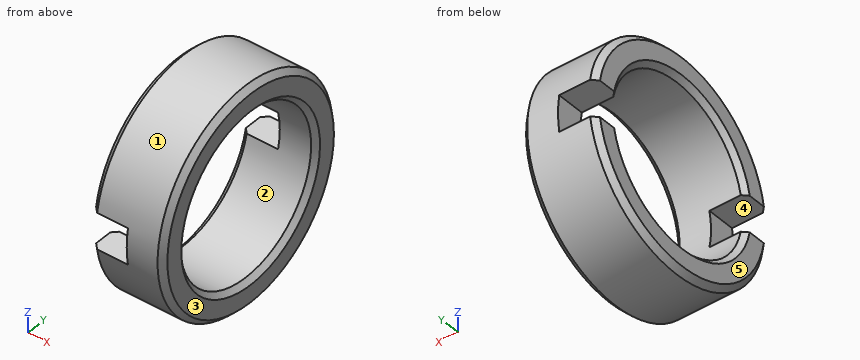
from build123d import *

# Parameters (mm, degrees)
CUT_EXTRUDE_1_DEPTH      = 1
CUT_EXTRUDE_1_DEPTH_BACK = 1
SKETCH_2_W               = 5
SKETCH_2_H               = 20


with BuildPart() as part:
    # 草图1 → 旋转1 (revolve)
    with BuildSketch(Plane.XY, mode=Mode.PRIVATE) as revolve_1_sk:
        Polygon((-2, 4.75), (-1.7295, 4.4795), (1.7295, 4.4795), (2, 4.75), (2, 5.7), (1.7, 6), (-1.7, 6), (-2, 5.7), align=None)
    revolve(revolve_1_sk.sketch.rotate(Axis((2, 0, 0), (-1, 0, 0)), 270), axis=Axis((2, 0, 0), (-1, 0, 0)))

    # 草图2 → 切除-拉伸1 (cut, two sides: drawn at the far end of the back side and taken through both)
    with BuildSketch(Plane.XY.offset(-CUT_EXTRUDE_1_DEPTH_BACK)):
        with Locations((-2.5, 0)):
            Rectangle(SKETCH_2_W, SKETCH_2_H)
    extrude(amount=CUT_EXTRUDE_1_DEPTH + CUT_EXTRUDE_1_DEPTH_BACK, mode=Mode.SUBTRACT)


solid = part.part
Work out the finished part from the listing and answer in its coordinate system (mm). Face numbers are marked on the shaded views. A direction names the side the tool comes from. Round coordinates to 2 decimals unless told otherwise and drop trailing zeros. Write each loop counter-clockwise with the first axis right and the second up, starting at its lowest first coordinate (ties: lowest second). Pieces come first, ordered by that corner, then holes. Notation, with made-up numbers: (82.25, 27.25) - (118.25, 27.25) arc R11 ccw to (118.25, 42.25) - close; hole circle Ø1 at (-29, -0.75). An arc over 180 degrees is marked (long way). Answer in a Markdown table with one row per item. Add a question column.
1. The mould has two halves that part along Z. Classify the marked faces 1, 2 and 3: +Z half, -Z half, draft (parallel to the pull), parting line (faces both ways), or undercut.
2. Find the intervals of material crossed by line 1 along Y through (x, z) = (0.8, 0); line 2 along Y through (x, z) = (-0.45, 1.75); line 3 along Z through (x, y) = (1.6, -0.5), in increasing order. Write a range as from..to.
3. For the marked faces 4 and 5, determine the directions among +Z, -Z, +X, -X, +Y, -Y from which every point of the face is accessible in a straight line to the end or side of a thin tool.
4. A cutting plane is placed at C-C, the plane y = 0. Determine the outline of the cut face in (x, z).
5. A cutting plane is placed at B-B, the plane x = -1.45. Determine the outline of the cut face in (y, z), and give its area (3 significant figures).
6. A cutting plane is placed at A-A, the plane z = 0. Determine the outline of the cut face in (x, y), and give its area (3 significant figures).
7. Given pin 1 (1.3 mm diameter, centred on y = 5, z = 0, fed in from -X); pin 2 (1 mm diameter, centred on x = 1.5, z = -1, fed in from -Y); pin 3 (1.2 mm diameter, centred on x = -1, y = 5, fed in from +Z), each flat-ended and moving along its own axis, determine where each tip first touches the part or whether it passes through.
Worked out:
| question | item | result |
|---|---|---|
| 1 | face 1 | parting line |
| 1 | face 2 | undercut |
| 1 | face 3 | draft |
| 2 | line 1 | -6..-4.48, 4.48..6 |
| 2 | line 2 | -5.74..-4.12, 4.12..5.74 |
| 2 | line 3 | -5.98..-4.45, 4.45..5.98 |
| 3 | face 4 | -X, +Y, -Y |
| 3 | face 5 | +Z, -Z, -X, +Y, -Y |
| 4 | outline | (-2, -5.7) - (-1.7, -6) - (1.7, -6) - (2, -5.7) - (2, -4.75) - (1.73, -4.48) - (-1.73, -4.48) - (-2, -4.75) - close; (-2, 4.75) - (-1.73, 4.48) - (1.73, 4.48) - (2, 4.75) - (2, 5.7) - (1.7, 6) - (-1.7, 6) - (-2, 5.7) - close |
| 5 | outline | (-5.92, -1) arc R6 ccw to (5.92, -1) - (4.37, -1) arc R4.48 cw to (-4.37, -1) - close; (-5.92, 1) - (-4.37, 1) arc R4.48 cw to (4.37, 1) - (5.92, 1) arc R6 ccw to start |
| 5 | area | 43.9 mm^2 |
| 6 | outline | (0, -6) - (1.7, -6) - (2, -5.7) - (2, -4.75) - (1.73, -4.48) - (0, -4.48) - close; (0, 4.48) - (1.73, 4.48) - (2, 4.75) - (2, 5.7) - (1.7, 6) - (0, 6) - close |
| 6 | area | 5.92 mm^2 |
| 7 | pin 1 | x = 0 |
| 7 | pin 2 | y = -5.98 |
| 7 | pin 3 | z = 4.08 |
